```python
from build123d import *

# Parameters (mm, degrees)
SKETCH_1_R          = 20
SKETCH_1_R_2        = 10
EXTRUDE_1_DEPTH     = 15
SKETCH_2_W          = 9.046336772
SKETCH_2_H          = 38.953764593
CUT_EXTRUDE_1_DEPTH = 33.015621187
CHAMFER_1_SIZE      = 1
SKETCH_3_W          = 2.1
SKETCH_3_H          = 20


with BuildPart() as part:
    # 草图1 → 凸台-拉伸1 (new body)
    with BuildSketch(Plane(origin=(0, 0, 0), x_dir=(1, 0, 0), z_dir=(0, 1, 0))):
        with Locations(Location((0, 0, 0), (0, 0, 270))):
            Circle(SKETCH_1_R)
        with Locations(Location((0, 0, 0), (0, 0, 270))):
            Circle(SKETCH_1_R_2, mode=Mode.SUBTRACT)
    extrude(amount=EXTRUDE_1_DEPTH)

    # 草图2 → 切除-拉伸1 (cut, through all)
    with BuildSketch(Plane(origin=(0, 15, 0), x_dir=(1, 0, 0), z_dir=(0, 1, 0))):
        with Locations((-19.523168386, 4.341186033)):
            Rectangle(SKETCH_2_W, SKETCH_2_H)
    extrude(amount=-CUT_EXTRUDE_1_DEPTH, mode=Mode.SUBTRACT)

    # 倒角1
    chamfer_1_edges = [part.edges().sort_by_distance(p)[0] for p in [
        (20, 15, 0),
        (20, 0, 0),
        (-15, 0, 0),
        (-15, 15, 0),
        (0, 0, -10),
        (0, 15, -10),
    ]]
    chamfer(chamfer_1_edges, length=CHAMFER_1_SIZE)

    # 草图3 → M5 螺纹孔1 (revolve, cut)
    with BuildSketch(Plane.ZX.offset(7.5)):
        with Locations((1.05, 10)):
            Rectangle(SKETCH_3_W, SKETCH_3_H)
    revolve(axis=Axis((-6.35, 7.5, 0), (1, 0, 0)), mode=Mode.SUBTRACT)


solid = part.part
```
CAD build for the part. Positions are in the model's coordinates, mm. A direction names the side the tool comes from. Coordinates: 2 decimals unless noted, no trailing zeros. Write each loop counter-clockwise with the first axis right and the second up, starting at its lowest first coordinate (ties: lowest second). Pieces come first, ordered by that corner, then holes. Notation, with made-up numbers: (73, 1) -> (104, 1) arc R18 cw to (104, 33) -> close; hole circle Ø4 at (-9.75, 88.5). An arc over 180 degrees is marked (long way). Return JSON: item names as keys, results as strings. Group by question number.
Q1. Pull direction Z, two halves, no side cores. Call faces 1 (the face through (19.15, 14.84, -0.65)), 2 (the face through (10, 0, 8)), 3 (the face through (-9.76, 7.41, -2.17)): released by +Z, released by -Z, zero draft, split by the parting line, or undercut.
Q2. Cut at D-D, the plane y = 7.5. Give the cut face in (x, z), then the cut area to 3 significant figures.
Q3. Drill centre lines: line 1 (X direction, y = 2.5, z = 0); line 2 (Y direction, x = 14.75, z = 0); line 3 (Z direction, x = -3.5, y = 14). Where is each one in solid material? Low to high.
Q4. Cut at C-C, the plane y = 13.25. Give the cut face in (x, z), then the cut area to 3 significant figures.
Q5. Cut at B-B, the plane x = 0. Give the cut face in (y, z), then the cut area to 3 significant figures.
Q6. Flat gauge pins, fed straight in: pin 1 (2 mm diameter, centred on y = 1.5, z = 8.5, fed in from +X); pin 2 (3 mm diameter, centred on x = -6.5, y = 9.5, fed in from -Z). Where does each tip first touch, or does it go through?
Q7. Which spindle directions (+Z, -Z, +X, -X, +Y, -Y) get a long thin tool onto all of the face, cutting with end or side? Do faces 4 (the face through (19.99, 4.52, 0.68)), 5 (the face through (14.957, 5.418, -0.273)). Say none if no direction does.
Q8. Cut at A-A, the plane z = 0. Give the cut face in (x, y).
Returned:
{
 "1": {"face 1": "split by the parting line", "face 2": "zero draft", "face 3": "undercut"},
 "2": {"outline": "(-15, -13.23) arc R20 ccw to (19.89, -2.1) -> (9.78, -2.1) arc R10 cw (long way) to (9.78, 2.1) -> (19.89, 2.1) arc R20 ccw to (-15, 13.23) -> close", "area": "810 mm2"},
 "3": {"line 1": "x = -15 to -10, 10 to 20", "line 2": "y = 0 to 5.4, 9.6 to 15", "line 3": "z = -19.69 to -9.37, 9.37 to 19.69"},
 "4": {"outline": "(-15, -13.23) arc R20 ccw (long way) to (-15, 13.23) -> close; hole circle Ø20 at (0, 0)", "area": "852 mm2"},
 "5": {"outline": "(0, -19) -> (1, -20) -> (14, -20) -> (15, -19) -> (15, -11) -> (14, -10) -> (1, -10) -> (0, -11) -> close; (0, 11) -> (1, 10) -> (14, 10) -> (15, 11) -> (15, 19) -> (14, 20) -> (1, 20) -> (0, 19) -> close", "area": "296 mm2"},
 "6": {"pin 1": "stops at x = 18.54", "pin 2": "stops at z = -19.36"},
 "7": {"face 4": "+Y, -Y", "face 5": "+X"},
 "8": {"outline": "(-15, 1) -> (-14, 0) -> (-11, 0) -> (-10, 1) -> (-10, 14) -> (-11, 15) -> (-14, 15) -> (-15, 14) -> close; (10, 1) -> (11, 0) -> (19, 0) -> (20, 1) -> (20, 5.4) -> (10, 5.4) -> close; (10, 9.6) -> (20, 9.6) -> (20, 14) -> (19, 15) -> (11, 15) -> (10, 14) -> close"}
}
